from build123d import *

# Parameters (mm, degrees)
SIDE_PROFILE_SKETCH_W            = 120
SIDE_PROFILE_SKETCH_H            = 10
MAIN_BODY_EXTRUDE_100_DEPTH      = 100
UPRIGHT_START                    = 5
SKETCH1_5_R                      = 2.5
SKETCH1_5_W                      = 120
SKETCH1_5_H                      = 80
SKETCH1_5_R_2                    = 4
UPRIGHT_BLOCK_EXTRUDE_35_DEPTH   = 35
FRONT_START                      = 5
SKETCH1_6_R                      = 2.5
FRONT_LEVER_ARM_EXTRUDE_10_DEPTH = 10
REAR_START                       = 60
SKETCH1_7_W                      = 120
SKETCH1_7_H                      = 70
REAR_LEVER_ARM_EXTRUDE_10_DEPTH  = 10


with BuildPart() as part:
    # Side Profile Sketch → Main Body Extrude 100 (new body)
    with BuildSketch(Plane.XY):
        with Locations((0, -35)):
            Rectangle(SIDE_PROFILE_SKETCH_W, SIDE_PROFILE_SKETCH_H)
    extrude(amount=MAIN_BODY_EXTRUDE_100_DEPTH)

    # Sketch1_5 → Upright Block Extrude 35 (add)
    # profile 1 of 3: a face of its own
    with BuildSketch(Plane.XY.offset(UPRIGHT_START)):
        with Locations((-105, 83.784559584)):
            Circle(SKETCH1_5_R)
    # profile 2 of 3: a face of its own
    with BuildSketch(Plane.XY.offset(UPRIGHT_START)):
        with Locations((105, 83.784559584)):
            Circle(SKETCH1_5_R)
    # profile 3 of 3: a face of its own
    with BuildSketch(Plane.XY.offset(UPRIGHT_START)):
        Rectangle(SKETCH1_5_W, SKETCH1_5_H)
        with Locations((-30, 0)):
            Circle(SKETCH1_5_R_2, mode=Mode.SUBTRACT)
        with Locations((30, 0)):
            Circle(SKETCH1_5_R_2, mode=Mode.SUBTRACT)
    extrude(amount=UPRIGHT_BLOCK_EXTRUDE_35_DEPTH)


with BuildPart() as upright_block_extrude_35_kept_piece:
    # of the separate pieces the step leaves, the one the design keeps (upright_block_extrude_35_pieces_kept)
    add(part.part.solids().sort_by_distance((60, -30, 0))[0])

    # Sketch1_6 → Front Lever Arm Extrude 10 (add)
    # profile 1 of 2: a face of its own
    with BuildSketch(Plane.XY.offset(FRONT_START)):
        with BuildLine():
            Line((102.433113428, 88.075374579), (30, 40))
            Line((30, 40), (60, 40))
            Line((60, 40), (109.439765001, 81.484888578))
            ThreePointArc((109.439765001, 81.484888578), (108.425718149, 87.426599557), (102.433113428, 88.075374579))
        make_face()
        with Locations((105, 83.784559584)):
            Circle(SKETCH1_6_R, mode=Mode.SUBTRACT)
    # profile 2 of 2: a face of its own
    with BuildSketch(Plane.XY.offset(FRONT_START)):
        with BuildLine():
            Line((-109.439765001, 81.484888578), (-60, 40))
            Line((-60, 40), (-30, 40))
            Line((-30, 40), (-102.433113428, 88.075374579))
            ThreePointArc((-102.433113428, 88.075374579), (-108.425718149, 87.426599557), (-109.439765001, 81.484888578))
        make_face()
        with Locations((-105, 83.784559584)):
            Circle(SKETCH1_6_R, mode=Mode.SUBTRACT)
    extrude(amount=FRONT_LEVER_ARM_EXTRUDE_10_DEPTH)

    # Sketch1_7 → Rear Lever Arm Extrude 10 (add)
    with BuildSketch(Plane.XY.offset(REAR_START)):
        with Locations((0, 5)):
            Rectangle(SKETCH1_7_W, SKETCH1_7_H)
    extrude(amount=REAR_LEVER_ARM_EXTRUDE_10_DEPTH)


solid = upright_block_extrude_35_kept_piece.part
Source: CAD feature listing. Evaluate the final solid. Frame: model axes, mm. A direction names the side the tool comes from. Round coordinates to 2 decimals unless told otherwise and drop trailing zeros. Order: outer loops, then holes, each group sorted by start corner. A loop starts at its lowest first (then second) coordinate and runs counter-clockwise, first axis right, second up. Notation, with made-up numbers: (-7, 55) -> (25, 55) arc R17 cw to (25, 72) -> close; hole circle Ø10 at (-21.75, 67). An arc over 180 degrees is marked (long way). Answer as CSV lines item,"result".
Item 1: Section D-D, the plane x = -1. Return loops of the section in (y, z), plus the area to 3 significant figures.
A:
outline,"(-40, 0) -> (-30, 0) -> (-30, 5) -> (40, 5) -> (40, 40) -> (-30, 40) -> (-30, 60) -> (40, 60) -> (40, 70) -> (-30, 70) -> (-30, 100) -> (-40, 100) -> close"
area,"4,150 mm²"
Item 2: Section B-B, the plane y = 31. Return loops of the section in (x, z).
A:
outline,"(-60, 5) -> (60, 5) -> (60, 40) -> (-60, 40) -> close; (-60, 60) -> (60, 60) -> (60, 70) -> (-60, 70) -> close"
Item 3: Line query: L1, parallel to Z at x = 4, y = 13.5; L2, parallel to Y at x = 7.5, z = 96.5; L3, parallel to X at y = -12, z = 10.5. Output: solid intervals per line, ascending.
A:
L1,"5 to 40, 60 to 70"
L2,"-40 to -30"
L3,"-60 to 60"
Item 4: Section A-A, the plane y = 0. Return loops of the section in (x, z), plus the area to 3 significant figures.
A:
outline,"(-60, 5) -> (-34, 5) -> (-34, 40) -> (-60, 40) -> close; (-60, 60) -> (60, 60) -> (60, 70) -> (-60, 70) -> close; (-26, 5) -> (26, 5) -> (26, 40) -> (-26, 40) -> close; (34, 5) -> (60, 5) -> (60, 40) -> (34, 40) -> close"
area,"4,840 mm²"
Item 5: Pull-direction query (Y, two-part tool) for faces 6 (the face through (-73, 59, 15)), 7 (the face through (-33.2, -2.4, 22.3)), 8 (the face through (-65.71, 63.7, 9.93)); classes: pulls with the +Y half, pulls with the -Y half, needs draft (parallel to the pull), parting line crosses it, or undercut.
A:
face 6,"needs draft"
face 7,"undercut"
face 8,"pulls with the +Y half"
Item 6: Pin query (flat end, axial travel): pin 1 Ø1 at (y, z) = (-27, 22) entering from +X; pin 2 Ø22 at (x, z) = (-24.5, 50.5) entering from +Y; pin 3 Ø8 at (x, y) = (105, 83.78) entering from -Z. Return the tip coordinate at first contact, or that it passes through.
A:
pin 1,"x = 60"
pin 2,"y = 40"
pin 3,"z = 5"
Item 7: Section C-C, the plane z = 18. Return loops of the section in (x, y), plus the area to 3 significant figures.
A:
outline,"(-60, -40) -> (60, -40) -> (60, 40) -> (-60, 40) -> close; hole circle Ø8 at (-30, 0); hole circle Ø8 at (30, 0)"
area,"9,500 mm²"
Item 8: Reachability of faces 1 (the face through (-1, 5, 40)), 2 (the face through (-1, -30, 2)), 3 (the face through (66.72, 64.37, 9.93)), 4 (the face through (-1, -35, 0)), 5 (the face through (73, 61, 15)) from +Z, -Z, +X, -X, +Y, -Y: full face, straight path, thin tool, end or side. Return the list, or none.
A:
face 1,"+X, -X, +Y"
face 2,"-Z, +X, -X, +Y"
face 3,"+Z, -Z, +Y"
face 4,"-Z, +X, -X, +Y, -Y"
face 5,"+Z, +X, -X, +Y"
